Design review of the part built by this model. Coordinates are the model's own, in mm. Face numbers are marked on the shaded views. Coordinates: 2 decimals unless noted, no trailing zeros. Write each loop counter-clockwise with the first axis right and the second up, starting at its lowest first coordinate (ties: lowest second). Pieces come first, ordered by that corner, then holes. Notation, with made-up numbers: (37.5, 77) - (54.5, 77) arc R28 cw to (54.5, 100) - close; hole circle Ø3 at (-22.5, -12.5). An arc over 180 degrees is marked (long way). One line per item, written item: value.
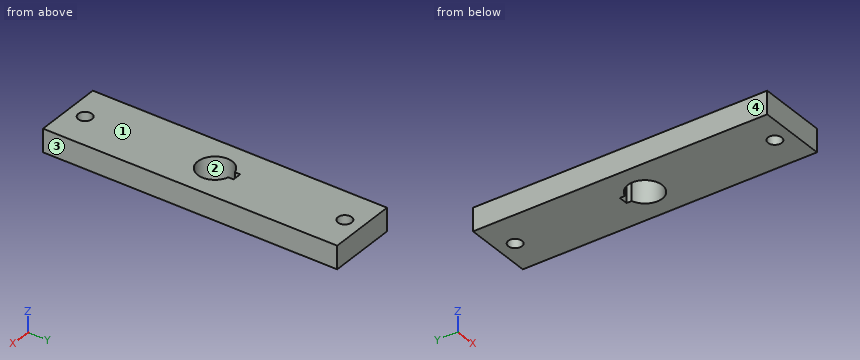
from build123d import *

# Parameters (mm, degrees)
SKETCH_1_W          = 60
SKETCH_1_H          = 256
EXTRUDE_1_DEPTH     = 20
SKETCH_2_R          = 6
CUT_EXTRUDE_1_DEPTH = 133.981201679
CUT_EXTRUDE_2_DEPTH = 133.981201679


with BuildPart() as part:
    # 草图1 → 凸台-拉伸1 (new body)
    with BuildSketch(Plane.XY):
        Rectangle(SKETCH_1_W, SKETCH_1_H)
    extrude(amount=EXTRUDE_1_DEPTH)

    # 草图2 → 切除-拉伸1 (cut, through all)
    with BuildSketch(Plane.XY.offset(20)):
        with Locations((0, 113)):
            Circle(SKETCH_2_R)
        with Locations((0, -113)):
            Circle(SKETCH_2_R)
    extrude(amount=-CUT_EXTRUDE_1_DEPTH, mode=Mode.SUBTRACT)

    # 草图3 → 切除-拉伸2 (cut, through all)
    with BuildSketch(Plane.XY.offset(20)):
        with BuildLine():
            Line((-4, 19), (4, 19))
            Line((4, 19), (4, 14.456832295))
            ThreePointArc((4, 14.456832295), (0, -15), (-4, 14.456832295))
            Line((-4, 14.456832295), (-4, 19))
        make_face()
    extrude(amount=-CUT_EXTRUDE_2_DEPTH, mode=Mode.SUBTRACT)


solid = part.part
1. Consider section A-A, the plane x = 0. Write out the cut boundary in (y, z).
Answer block:
outline: (-128, 0) - (-119, 0) - (-119, 20) - (-128, 20) - close; (-107, 0) - (-15, 0) - (-15, 20) - (-107, 20) - close; (19, 0) - (107, 0) - (107, 20) - (19, 20) - close; (119, 0) - (128, 0) - (128, 20) - (119, 20) - close
2. Consider section B-B, the plane y = 12. Write out the cut boundary in (x, z).
Answer block:
outline: (-30, 0) - (-9, 0) - (-9, 20) - (-30, 20) - close; (9, 0) - (30, 0) - (30, 20) - (9, 20) - close
3. Mouldability with a two-part tool opening along X and no side actions: class the marked faces 1, 2, 3 and 4 as released by +X, released by -X, zero draft, split by the parting line, or undercut.
Answer block:
face 1: zero draft
face 2: undercut
face 3: released by +X
face 4: released by -X
4. Wall thickness on line 1 along Y through (x, z) = (0, 5); line 2 along Y through (x, z) = (5.5, 15.5); line 3 along X through (y, z) = (-1, 11): over which ranges is each line inside the solid? List them lowest first.
Answer block:
line 1: y = -128 to -119, -107 to -15, 19 to 107, 119 to 128
line 2: y = -128 to -115.4, -110.6 to -13.96, 13.96 to 110.6, 115.4 to 128
line 3: x = -30 to -14.97, 14.97 to 30
5. Consider section C-C, the plane z = 4.75. Write out the cut boundary in (x, y), then the cut area to 3 significant figures.
Answer block:
outline: (-30, -128) - (30, -128) - (30, 128) - (-30, 128) - close; hole circle Ø12 at (0, -113); hole circle Ø12 at (0, 113); hole (-4, 14.46) arc R15 ccw (long way) to (4, 14.46) - (4, 19) - (-4, 19) - close
area: 14,400 mm^2
6. Insertion check: pin 1 Ø15.5 at (x, y) = (0, -113) entering from +Z; pin 2 Ø7 at (x, y) = (0, 113) entering from -Z. Each pin has a flat end and moves straight along its axis. Give the tip position at first contact, or say it passes through.
Answer block:
pin 1: stops at z = 20
pin 2: passes through
7. Consider section D-D, the plane y = 113. Write out the cut boundary in (x, z).
Answer block:
outline: (-30, 0) - (-6, 0) - (-6, 20) - (-30, 20) - close; (6, 0) - (30, 0) - (30, 20) - (6, 20) - close
